Check sheet for the modelled part. Datum: model origin and axes. Units: mm. A direction names the side the tool comes from. Round coordinates to 2 decimals unless told otherwise and drop trailing zeros. Write each loop counter-clockwise with the first axis right and the second up, starting at its lowest first coordinate (ties: lowest second). Pieces come first, ordered by that corner, then holes. Notation, with made-up numbers: M -0.75,50.25 L 35.25,50.25 A25 ccw 35.25,67.25 Z; hole C -8.5,15 d5. An arc over 180 degrees is marked long. Put each result on its own line as item: value.
```python
from build123d import *


with BuildPart() as part:
    # 草图1 → 旋转1 (revolve)
    with BuildSketch(Plane.XY, mode=Mode.PRIVATE) as revolve_1_sk:
        Polygon((-0.9, 24.75), (0.9, 24.75), (0.9, 20.5), (24.5, 20.5), (24.5, 12.5), (25.5, 12.5), (25.5, 10), (-25.5, 10), (-25.5, 12.5), (-24.5, 12.5), (-24.5, 20.5), (-0.9, 20.5), align=None)
    revolve(revolve_1_sk.sketch.rotate(Axis((-73.221991318, 0, 0), (1, 0, 0)), 90), axis=Axis((-73.221991318, 0, 0), (1, 0, 0)))


solid = part.part
```
1. Access from +Z, -Z, +X, -X, +Y, -Y to the whole of each face (thin tool, end or side, straight path). Record for faces 1 (the cylindrical face through (0.01, -16.73, -18.24)), 2 (the cylindrical face through (12.865, 7.852, 18.937)), 3 (the cylindrical face through (-12.535, 7.852, 18.937)).
Computed values:
face 1: +X, -X
face 2: +X
face 3: -X
2. Cross-section at D-D (x = 4.5). Enter the section's corners in (y, z).
Computed values:
outline: C 0,0 d41; hole C 0,0 d20
3. Cross-section at A-A (y = 0). Enter the section's corners in (x, z).
Computed values:
outline: M -25.5,-12.5 L -24.5,-12.5 L -24.5,-20.5 L -0.9,-20.5 L -0.9,-24.75 L 0.9,-24.75 L 0.9,-20.5 L 24.5,-20.5 L 24.5,-12.5 L 25.5,-12.5 L 25.5,-10 L -25.5,-10 Z; M -25.5,10 L 25.5,10 L 25.5,12.5 L 24.5,12.5 L 24.5,20.5 L 0.9,20.5 L 0.9,24.75 L -0.9,24.75 L -0.9,20.5 L -24.5,20.5 L -24.5,12.5 L -25.5,12.5 Z
4. Scan lines: probe 1 along Y at (x, z) = (-15, 0); probe 2 along Y at (x, z) = (-0.5, 0); probe 3 along X at (y, z) = (12, 10.5). Record each from-to range of solid material in increasing order.
Computed values:
probe 1: y = -20.5 to -10, 10 to 20.5
probe 2: y = -24.75 to -10, 10 to 24.75
probe 3: x = -24.5 to 24.5
5. Release check for a two-part mould opening along Y. For faces 4 (the cylindrical face through (25.007, -3.755, 11.923)), 5 (the flat face through (-25.5, -10.2, 0.1)), 6 (the cylindrical face through (0, 0, -10)) record: +Y half, -Y half, draft (parallel to the pull), parting line (faces both ways), or undercut.
Computed values:
face 4: parting line
face 5: draft
face 6: undercut
6. Depth check by flat-ended pin: pin 1 Ø2 at (x, y) = (17.5, 6.5) entering from -Z; pin 2 Ø4 at (x, z) = (-19.5, -12) entering from -Y; pin 3 Ø10 at (x, z) = (-2.5, -7.5) entering from +Y; pin 4 Ø12.5 at (y, z) = (-2.5, -6.5) entering from -X. Enter the tip coordinate at first touch or a pass-through.
Computed values:
pin 1: stops at z = -19.75
pin 2: stops at y = -17.9
pin 3: stops at y = 24.6
pin 4: stops at x = -25.5
7. Cross-section at C-C (z = -14). Enter the section's corners in (x, y), then the cut area to 3 significant figures.
Computed values:
outline: M -24.5,-14.97 L -0.9,-14.97 L -0.9,-20.41 L 0.9,-20.41 L 0.9,-14.97 L 24.5,-14.97 L 24.5,14.97 L 0.9,14.97 L 0.9,20.41 L -0.9,20.41 L -0.9,14.97 L -24.5,14.97 Z
area: 1,490 mm2
